```python
from build123d import *

# Parameters (mm, degrees)
SKETCH_1_W            = 70
SKETCH_1_H            = 190
EXTRUDE_1_DEPTH       = 10
HOLE_WIZARD_M6_1_D    = 5
HOLE_WIZARD_9_0_9_1_D = 9
CHAMFER_1_SIZE        = 3


with BuildPart() as part:
    # 草图1 → 凸台-拉伸1 (new body)
    with BuildSketch(Plane(origin=(0, 0, 0), x_dir=(1, 0, 0), z_dir=(0, 1, 0))):
        Rectangle(SKETCH_1_W, SKETCH_1_H)
    extrude(amount=EXTRUDE_1_DEPTH)

    # M6 螺纹孔1 (through all)
    with Locations(Plane(origin=(0, 10, 0), x_dir=(1, 0, 0), z_dir=(0, 1, 0))):
        with Locations((18.5, 45), (-18.5, 45), (0, 45), (0, -45), (-18.5, -45), (18.5, -45)):
            Hole(HOLE_WIZARD_M6_1_D / 2)

    # Ø9.0 (9) 直径孔1 (through all)
    with Locations(Plane(origin=(0, 10, 0), x_dir=(1, 0, 0), z_dir=(0, 1, 0))):
        with Locations((-20, 77.5), (20, 77.5), (20, -77.5), (-20, -77.5)):
            Hole(HOLE_WIZARD_9_0_9_1_D / 2)

    # 倒角1
    chamfer_1_edges = [part.edges().sort_by_distance(p)[0] for p in [
        (35, 5, 95),
        (-35, 5, 95),
        (-35, 5, -95),
        (35, 5, -95),
    ]]
    chamfer(chamfer_1_edges, length=CHAMFER_1_SIZE)


solid = part.part
```
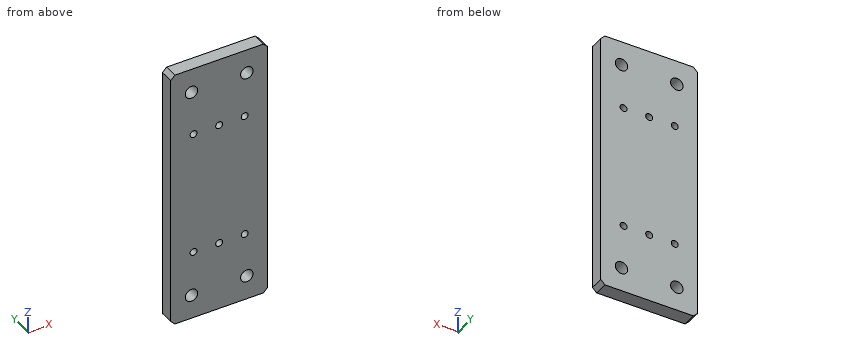
Source: CAD feature listing. Evaluate the final solid. Frame: model axes, mm. Round coordinates to 2 decimals unless told otherwise and drop trailing zeros. Write each loop counter-clockwise with the first axis right and the second up, starting at its lowest first coordinate (ties: lowest second). Pieces come first, ordered by that corner, then holes. Notation, with made-up numbers: M 84.5,-19 L 142.5,-19 A23 cw 142.5,13 Z; hole C 41,17.25 d5. An arc over 180 degrees is marked long. Use CSV: the item, a comma, the result in double quotes. Start each with the question number.
Q1. Cut plane D-D on z = -77.5. Output: boundary loops of the cut face in (x, y), plus the area to 3 significant figures.
Q2. Cut plane C-C on y = 4. Count the separate pieces of the cut face and the enclosed holes in it, plus the area to 3 significant figures.
Q3. Line query: line 1 (Z direction, x = 0, y = 3.25); line 2 (X direction, y = 6.75, z = -77.5); line 3 (X direction, y = 6, z = 75.5). Output: solid intervals per line, ascending. Write a range as from..to.
Q4. Cut plane B-B on x = 18.5. Output: boundary loops of the cut face in (y, z), plus the area to 3 significant figures.
Q5. Cut plane A-A on z = 45. Output: boundary loops of the cut face in (x, y), plus the area to 3 significant figures.
Results found:
1,outline,"M -35,0 L -24.5,0 L -24.5,10 L -35,10 Z; M -15.5,0 L 15.5,0 L 15.5,10 L -15.5,10 Z; M 24.5,0 L 35,0 L 35,10 L 24.5,10 Z"
1,area,"520 mm^2"
2,separate pieces,"1"
2,enclosed holes,"10"
2,area,"12,900 mm^2"
3,line 1,"-95..-47.5, -42.5..42.5, 47.5..95"
3,line 2,"-35..-24.5, -15.5..15.5, 24.5..35"
3,line 3,"-35..-24.03, -15.97..15.97, 24.03..35"
4,outline,"M 0,-95 L 10,-95 L 10,-81.74 L 0,-81.74 Z; M 0,-73.26 L 10,-73.26 L 10,-47.5 L 0,-47.5 Z; M 0,-42.5 L 10,-42.5 L 10,42.5 L 0,42.5 Z; M 0,47.5 L 10,47.5 L 10,73.26 L 0,73.26 Z; M 0,81.74 L 10,81.74 L 10,95 L 0,95 Z"
4,area,"1,630 mm^2"
5,outline,"M -35,0 L -21,0 L -21,10 L -35,10 Z; M -16,0 L -2.5,0 L -2.5,10 L -16,10 Z; M 2.5,0 L 16,0 L 16,10 L 2.5,10 Z; M 21,0 L 35,0 L 35,10 L 21,10 Z"
5,area,"550 mm^2"
